```python
from build123d import *

# Parameters (mm, degrees)
BASE_PLATE_SKETCH_R       = 6
BASE_PLATE_DEPTH          = 6
BEARING_UPRIGHT_SKETCH_R  = 15
BEARING_UPRIGHT_DEPTH     = 30
SUPPORT_RIB_10MM_REACH    = 152.552
SUPPORT_RIB_SKETCH_WALL_W = 425.186572672
SUPPORT_RIB_SKETCH_WALL_H = 10


with BuildPart() as part:
    # Base Plate Sketch → Base Plate (new, symmetric)
    with BuildSketch(Plane(origin=(0, 0, 0), x_dir=(1, 0, 0), z_dir=(0, 1, 0))):
        with BuildLine():
            Line((20, 25), (20, -25))
            ThreePointArc((20, -25), (0, -45), (-20, -25))
            Line((-20, -25), (-20, -15))
            Line((-20, -15), (-70, -15))
            Line((-70, -15), (-70, 15))
            Line((-70, 15), (-20, 15))
            Line((-20, 15), (-20, 25))
            ThreePointArc((-20, 25), (0, 45), (20, 25))
        make_face()
        with Locations(Location((0, 25, 0), (0, 0, 270))):
            Circle(BASE_PLATE_SKETCH_R, mode=Mode.SUBTRACT)
        with Locations(Location((0, -25, 0), (0, 0, 270))):
            Circle(BASE_PLATE_SKETCH_R, mode=Mode.SUBTRACT)
    extrude(amount=BASE_PLATE_DEPTH, both=True)

    # Bearing Upright Sketch → Bearing Upright (add, symmetric)
    with BuildSketch(Plane.XY):
        with BuildLine():
            Line((-70, -6), (-95, -6))
            Line((-95, -6), (-95, 19))
            ThreePointArc((-95, 19), (-97.235198346, 25.974858325), (-103.108108108, 30.351351351))
            ThreePointArc((-103.108108108, 30.351351351), (-109.530954843, 74.34333678), (-70, 54))
            Line((-70, 54), (-70, -6))
        make_face()
        with Locations((-95, 54)):
            Circle(BEARING_UPRIGHT_SKETCH_R, mode=Mode.SUBTRACT)
    extrude(amount=BEARING_UPRIGHT_DEPTH, both=True)

    # Support Rib Sketch wall → Support Rib 10mm (add, up to next)
    with BuildSketch(Plane(origin=(-30.468854155, 40.335036919, 0), x_dir=(-0.826802953509, 0.562491667554, 0), z_dir=(-0.562491667554, -0.826802953509, 0)), mode=Mode.PRIVATE) as support_rib_10mm_sk1:
        Rectangle(SUPPORT_RIB_SKETCH_WALL_W, SUPPORT_RIB_SKETCH_WALL_H)
    support_rib_10mm_tool1 = extrude(support_rib_10mm_sk1.sketch, amount=SUPPORT_RIB_10MM_REACH, mode=Mode.PRIVATE) - part.part
    add(support_rib_10mm_tool1.solids().sort_by_distance((-30.468854155, 40.335036919, 0))[0])


solid = part.part
```
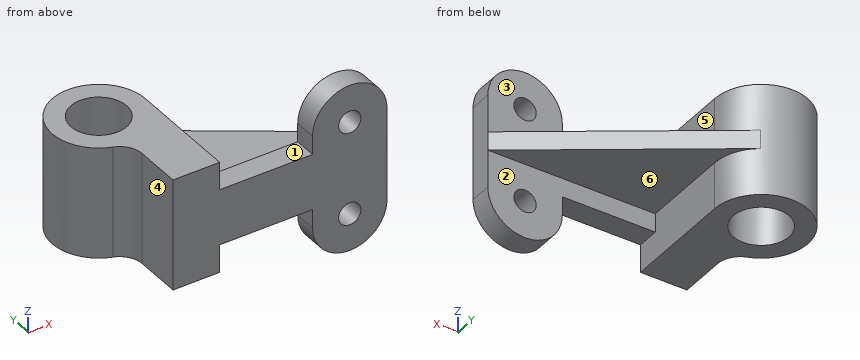
Build history of the part. All positions in model axes, mm. Face numbers are marked on the shaded views. A direction names the side the tool comes from. Round coordinates to 2 decimals unless told otherwise and drop trailing zeros. Loops run counter-clockwise (first coordinate to the right, second up) from the corner with the lowest first, then second, coordinate; pieces in that order, holes last.
Item 1: Saw through at B-B (z = 11.5). List the corners of the cut face in (x, y), then the cut area to 3 significant figures.
Item 2: Which spindle directions (+Z, -Z, +X, -X, +Y, -Y) get a long thin tool onto all of the face, cutting with end or side? Do the marked faces 1, 2 and 3. Say none if no direction does.
Item 3: Saw through at D-D (x = 0). List the corners of the cut face in (y, z), then the cut area to 3 significant figures.
Item 4: Two-plate mould, pull along X, no slides. Class the marked faces 4, 5 and 6: released by +X, released by -X, zero draft, split by the parting line, or undercut.
Item 5: Saw through at A-A (y = 3.5). List the corners of the cut face in (x, z), then the cut area to 3 significant figures.
Item 6: Drill centre lines: line 1 along X through (y, z) = (3, 25); line 2 along Y through (x, z) = (-21, -7.5); line 3 along X through (y, z) = (8, 6). Where is each one in solid material? Low to high.
Item 7: Pin check, flat tips, straight feed: P1, Ø1.5, axis at x = -91, y = 19, coming from the +Z side; P2, Ø6, axis at x = -102.5, z = 3.5, coming from the -Y side; P3, Ø12, axis at x = -37.5, y = 37.5, coming from the +Z side. Stop position of each tip, or through.
Item 8: Saw through at C-C (y = 45.5). List the corners of the cut face in (x, z), then the cut area to 3 significant figures.
Worked answers:
1. outline: (-103.11, 30.35) arc R12 cw to (-95, 19) - (-95, -6) - (20, -6) - (20, 6) - (-70, 6) - (-70, 54) arc R25 ccw (long way) to start; hole circle Ø30 at (-95, 54)
1. area: 3,360 mm2
2. face 1: +Z, +Y, -Y
2. face 2: -Z, +X, +Y
2. face 3: +Z, +X, +Y
3. outline: (-6, -45) - (6, -45) - (6, -31) - (-6, -31) - close; (-6, -19) - (6, -19) - (6, -5) - (19.61, -5) - (19.61, 5) - (6, 5) - (6, 19) - (-6, 19) - close; (-6, 31) - (6, 31) - (6, 45) - (-6, 45) - close
3. area: 928 mm2
4. face 4: released by -X
4. face 5: undercut
4. face 6: zero draft
5. outline: (-95, -30) - (-70, -30) - (-70, -15) - (-20, -15) - (-20, -25) arc R20 ccw to (20, -25) - (20, 25) arc R20 ccw to (-20, 25) - (-20, 15) - (-70, 15) - (-70, 30) - (-95, 30) - close; hole circle Ø12 at (0, -25); hole circle Ø12 at (0, 25)
5. area: 6,030 mm2
6. line 1: x = -95 to -70, -20 to -6, 6 to 20
6. line 2: y = -6 to 6
6. line 3: x = -95 to -70
7. P1: stops at z = 30
7. P2: stops at y = 28.37
7. P3: stops at z = 5
8. outline: (-118.51, -30) - (-107.36, -30) - (-107.36, 30) - (-118.51, 30) - close; (-82.64, -30) - (-70, -30) - (-70, -5) - (-38.06, -5) - (-38.06, 5) - (-70, 5) - (-70, 30) - (-82.64, 30) - close
8. area: 1,750 mm2
